```python
from build123d import *

# Parameters (mm, degrees)
HOLE_WIZARD_M4_1_D   = 3.3
SKETCH_4_OUTSIDE_W   = 67.858
SKETCH_4_OUTSIDE_H   = 67.858
SKETCH_4_OUTSIDE_W_2 = 45
SKETCH_4_OUTSIDE_H_2 = 45
CUT_EXTRUDE_1_DEPTH  = 10
CHAMFER_1_SIZE       = 0.5
SKETCH_5_W           = 1.1
SKETCH_5_H           = 0.35


with BuildPart() as part:
    # 草图1 → 旋转1 (revolve)
    with BuildSketch(Plane(origin=(0, 0, 0), x_dir=(1, 0, 0), z_dir=(0, 1, 0))):
        Polygon((0, 0), (0, 24), (5, 24), (5, 8.5), (9, 8.5), (9, 7.5), (47, 7.5), (47, 5), (58, 5), (58, 0), align=None)
    revolve(axis=Axis((58, 0, 0), (-1, 0, 0)))

    # M4 螺纹孔1 (through all)
    with Locations(Plane(origin=(0, 13.5, -15), x_dir=(0, 0, -1), z_dir=(-1, 0, 0))):
        with Locations((0, 0), (-30, 0), (0, 27), (-30, 27)):
            Hole(HOLE_WIZARD_M4_1_D / 2)

    # 草图4 outside → 切除-拉伸1 (cut)
    with BuildSketch(Plane.ZY):
        Rectangle(SKETCH_4_OUTSIDE_W, SKETCH_4_OUTSIDE_H)
        Rectangle(SKETCH_4_OUTSIDE_W_2, SKETCH_4_OUTSIDE_H_2, mode=Mode.SUBTRACT)
    extrude(amount=-CUT_EXTRUDE_1_DEPTH, mode=Mode.SUBTRACT)

    # 倒角1
    chamfer_1_edges = [part.edges().sort_by_distance(p)[0] for p in [
        (58, 0, 5),
        (47, 0, 7.5),
    ]]
    chamfer(chamfer_1_edges, length=CHAMFER_1_SIZE)

    # 草图5 → 切除-旋转1 (revolve, cut)
    with BuildSketch(Plane(origin=(0, 0, 0), x_dir=(1, 0, 0), z_dir=(0, 1, 0))):
        with Locations((44.55, 7.325)):
            Rectangle(SKETCH_5_W, SKETCH_5_H)
    revolve(axis=Axis((0, 0, 0), (1, 0, 0)), mode=Mode.SUBTRACT)


solid = part.part
```
Build history of the part. All positions in model axes, mm. A direction names the side the tool comes from. Coordinates: 2 decimals unless noted, no trailing zeros. Write each loop counter-clockwise with the first axis right and the second up, starting at its lowest first coordinate (ties: lowest second). Pieces come first, ordered by that corner, then holes.
1. 3-axis set-ups, long thin cutter, end or side, ignore diameter. For faces 4 (the cylindrical face through (44.56, 7.09, 0.93)), 5 (the cylindrical face through (2.535, 13.004, 16.574)), 6 (the cylindrical face through (7.028, -7.167, -4.57)): which of +Z, -Z, +X, -X, +Y, -Y reach the whole face in a straight line?
Answer block:
face 4: none
face 5: +X, -X
face 6: +X
2. Drill centre lines: probe 1 along Y at (x, z) = (1, -15) (3 decimals); probe 2 along X at (y, z) = (5.5, 18.5); probe 3 along Z at (x, y) = (1.9, -13.5). Where is each one in solid material? Low to high.
Answer block:
probe 1: y = -18.735 to -15.15, -11.85 to 11.85, 15.15 to 18.735
probe 2: x = 0 to 5
probe 3: z = -19.84 to -16.65, -13.35 to 13.35, 16.65 to 19.84
3. Drop flat-ended pins along their axis: pin 1 (6 mm diameter, centred on y = 10, z = 17.5, fed in from +X); pin 2 (2 mm diameter, centred on x = 49, z = -1.5, fed in from +Y); pin 3 (4 mm diameter, centred on x = 50.5, z = 3.5, fed in from -Y). Give the stop position or say it passes through.
Answer block:
pin 1: stops at x = 5
pin 2: stops at y = 4.97
pin 3: stops at y = -4.77
4. Band-saw the part on B-B, the plane z = 0. Give the cut face in (x, y), and give its area (3 significant figures).
Answer block:
outline: (0, -22.5) - (5, -22.5) - (5, -8.5) - (9, -8.5) - (9, -7.5) - (44, -7.5) - (44, -7.15) - (45.1, -7.15) - (45.1, -7.5) - (46.5, -7.5) - (47, -7) - (47, -5) - (57.5, -5) - (58, -4.5) - (58, 4.5) - (57.5, 5) - (47, 5) - (47, 7) - (46.5, 7.5) - (45.1, 7.5) - (45.1, 7.15) - (44, 7.15) - (44, 7.5) - (9, 7.5) - (9, 8.5) - (5, 8.5) - (5, 22.5) - (0, 22.5) - close
area: 972 mm2
5. Band-saw the part on A-A, the plane y = 13.5. Give the cut face in (x, z).
Answer block:
outline: (0, -19.84) - (5, -19.84) - (5, -16.65) - (0, -16.65) - close; (0, -13.35) - (5, -13.35) - (5, 13.35) - (0, 13.35) - close; (0, 16.65) - (5, 16.65) - (5, 19.84) - (0, 19.84) - close
6. Band-saw the part on D-D, the plane z = -15. Give the cut face in (x, y) (3 decimals).
Answer block:
outline: (0, -18.735) - (5, -18.735) - (5, -15.15) - (0, -15.15) - close; (0, -11.85) - (5, -11.85) - (5, 11.85) - (0, 11.85) - close; (0, 15.15) - (5, 15.15) - (5, 18.735) - (0, 18.735) - close
7. Pull direction Z, two halves, no side cores. Call faces 1 (the cylindrical face through (52.32, 4.88, 1.08)), 2 (the flat face through (9, 8, 0)), 3 (the cylindrical face through (2.535, 14.132, -13.476)): released by +Z, released by -Z, zero draft, split by the parting line, or undercut.
Answer block:
face 1: split by the parting line
face 2: zero draft
face 3: undercut
